Could you check a few things on this model? Use its own coordinates, in mm. Face numbers are marked on the shaded views. A direction names the side the tool comes from. Round coordinates to 2 decimals unless told otherwise and drop trailing zeros. Write each loop counter-clockwise with the first axis right and the second up, starting at its lowest first coordinate (ties: lowest second). Pieces come first, ordered by that corner, then holes. Notation, with made-up numbers: (54.5, -14) -> (64.5, -14) arc R17 ccw to (64.5, -7) -> close; hole circle Ø2 at (31.5, 70). An arc over 180 degrees is marked (long way). Answer in a Markdown table with one row per item. Add a question column.
```python
from build123d import *

# Parameters (mm, degrees)
BRACKET_BODY_DEPTH     = 50
POCKET_SKETCH_W        = 8
POCKET_SKETCH_H        = 60
POCKET_60X30_DEPTH     = 433.810582126
RAISED_PAD_SKETCH_R    = 25
RAISED_PAD_5MM_DEPTH   = 5
PAD_HOLE_SKETCH_R      = 10
PAD_HOLES_DEPTH        = 328.146756059
MOUNTING_HOLE_SKETCH_R = 7.25
MOUNTING_HOLES_DEPTH   = 25
THROUGH_HOLE_SKETCH_R  = 8
THROUGH_HOLES_16_DEPTH = 20
SADDLE_BLOCK_DEPTH     = 55
PIPE_SADDLE_CUT_DEPTH  = 55
SUPPORT_ARM_DEPTH      = 25
SUPPORT_WEB_15MM_DEPTH = 7.5


with BuildPart() as part:
    # Bracket Profile Sketch → Bracket Body (new, symmetric)
    with BuildSketch(Plane.XY):
        with BuildLine():
            Line((0, 110), (0, -250))
            Line((0, -250), (-25, -250))
            Line((-25, -250), (-25, -45))
            ThreePointArc((-25, -45), (-30.857864376, -30.857864376), (-45, -25))
            Line((-45, -25), (-235, -25))
            Line((-235, -25), (-235, 0))
            Line((-235, 0), (-45, 0))
            ThreePointArc((-45, 0), (-30.857864376, 5.857864376), (-25, 20))
            Line((-25, 20), (-25, 110))
            Line((-25, 110), (0, 110))
        make_face()
    extrude(amount=BRACKET_BODY_DEPTH, both=True)

    # Pocket Sketch → Pocket 60x30 (cut, through all)
    with BuildSketch(Plane(origin=(0, 110, 0), x_dir=(1, 0, 0), z_dir=(0, 1, 0))):
        with Locations((-4, 0)):
            Rectangle(POCKET_SKETCH_W, POCKET_SKETCH_H)
    extrude(amount=-POCKET_60X30_DEPTH, mode=Mode.SUBTRACT)

    # Raised Pad Sketch → Raised Pad 5mm (add)
    with BuildSketch(Plane.ZY.offset(25)):
        with Locations(Location((0, 75, 0), (0, 0, 90))):
            Circle(RAISED_PAD_SKETCH_R)
        with Locations(Location((0, -215, 0), (0, 0, 180))):
            Circle(RAISED_PAD_SKETCH_R)
    extrude(amount=RAISED_PAD_5MM_DEPTH)

    # Pad Hole Sketch → Pad Holes (cut, through all)
    with BuildSketch(Plane.ZY.offset(30)):
        with Locations(Location((0, 75, 0), (0, 0, 270))):
            Circle(PAD_HOLE_SKETCH_R)
        with Locations(Location((0, -215, 0), (0, 0, 270))):
            Circle(PAD_HOLE_SKETCH_R)
    extrude(amount=-PAD_HOLES_DEPTH, mode=Mode.SUBTRACT)

    # Mounting Hole Sketch → Mounting Holes (cut)
    with BuildSketch(Plane(origin=(0, 0, 0), x_dir=(1, 0, 0), z_dir=(0, 1, 0))):
        with Locations(Location((-75, 0, 0), (0, 0, 270))):
            Circle(MOUNTING_HOLE_SKETCH_R)
        with Locations(Location((-215, 0, 0), (0, 0, 270))):
            Circle(MOUNTING_HOLE_SKETCH_R)
    extrude(amount=-MOUNTING_HOLES_DEPTH, mode=Mode.SUBTRACT)

    # Through Hole Sketch → Through Holes Ø16 (cut)
    with BuildSketch(Plane(origin=(0, 0, 0), x_dir=(1, 0, 0), z_dir=(0, 1, 0))):
        with Locations(Location((-75, 0, 0), (0, 0, 270))):
            Circle(THROUGH_HOLE_SKETCH_R)
        with Locations(Location((-215, 0, 0), (0, 0, 270))):
            Circle(THROUGH_HOLE_SKETCH_R)
    extrude(amount=-THROUGH_HOLES_16_DEPTH, mode=Mode.SUBTRACT)

    # Saddle Block Sketch → Saddle Block (add, symmetric)
    with BuildSketch(Plane.XY):
        with BuildLine():
            Line((-194.749371855, 0), (-95.250628145, 0))
            ThreePointArc((-95.250628145, 0), (-145, -55), (-194.749371855, 0))
        make_face()
    extrude(amount=SADDLE_BLOCK_DEPTH, both=True)

    # Pipe Saddle Cut Sketch → Pipe Saddle Cut (cut, symmetric)
    with BuildSketch(Plane.XY):
        with BuildLine():
            Line((-190, 0), (-100, 0))
            Line((-100, 0), (-100, -5))
            Line((-100, -5), (-105, -5))
            ThreePointArc((-105, -5), (-145, -45), (-185, -5))
            Line((-185, -5), (-190, -5))
            Line((-190, -5), (-190, 0))
        make_face()
    extrude(amount=PIPE_SADDLE_CUT_DEPTH, both=True, mode=Mode.SUBTRACT)

    # Support Arm Sketch → Support Arm (add, symmetric)
    with BuildSketch(Plane.XY):
        with BuildLine():
            Line((-41.449496417, -158.46530057), (-175.781812899, -109.572335871))
            ThreePointArc((-175.781812899, -109.572335871), (-218.723683986, -76.621879272), (-235, -25))
            Line((-235, -25), (-219.833147735, -25))
            ThreePointArc((-219.833147735, -25), (-223.484631452, -26.584349745), (-224.822024251, -30.333333333))
            ThreePointArc((-224.822024251, -30.333333333), (-208.965317539, -73.046208509), (-172.361611466, -100.175409663))
            Line((-172.361611466, -100.175409663), (-42.446261863, -147.460729893))
            ThreePointArc((-42.446261863, -147.460729893), (-30.543506327, -145.893702398), (-25, -135.244725822))
            Line((-25, -135.244725822), (-25, -181.95761609))
            ThreePointArc((-25, -181.95761609), (-29.521198893, -167.618205181), (-41.449496417, -158.46530057))
        make_face()
    extrude(amount=SUPPORT_ARM_DEPTH, both=True)

    # Support Web Sketch → Support Web 15mm (add, symmetric)
    with BuildSketch(Plane.XY):
        with BuildLine():
            Line((-25, -45), (-25, -135.244725822))
            ThreePointArc((-25, -135.244725822), (-30.543506327, -145.893702398), (-42.446261863, -147.460729893))
            Line((-42.446261863, -147.460729893), (-172.361611466, -100.175409663))
            ThreePointArc((-172.361611466, -100.175409663), (-208.965317539, -73.046208509), (-224.822024251, -30.333333333))
            ThreePointArc((-224.822024251, -30.333333333), (-223.484631452, -26.584349745), (-219.833147735, -25))
            Line((-219.833147735, -25), (-190.82575695, -25))
            ThreePointArc((-190.82575695, -25), (-145, -55), (-99.17424305, -25))
            Line((-99.17424305, -25), (-45, -25))
            ThreePointArc((-45, -25), (-30.857864376, -30.857864376), (-25, -45))
        make_face()
    extrude(amount=SUPPORT_WEB_15MM_DEPTH, both=True)


solid = part.part
```
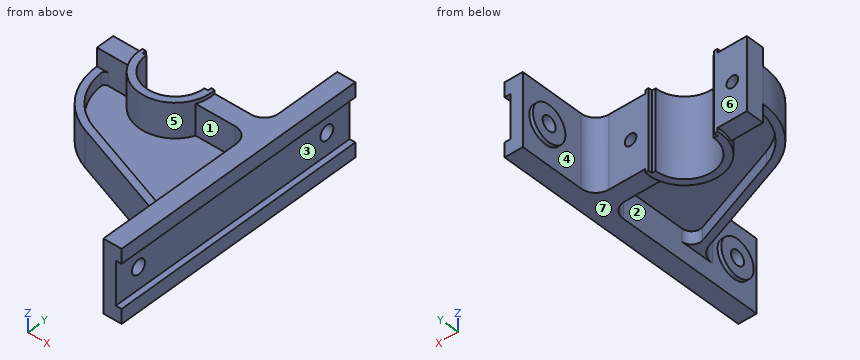
(1) I need wall thicknesses on L1, parallel to X at y = -4.75, z = 0; L2, parallel to Z at x = -215, y = -21.65; L3, parallel to X at y = -22.2, z = 0. Which ranges of each line are inside material? Lowest first, please.
(2) For P1, Ø8, axis at x = -190, z = 7, coming from the +Y side; P2, Ø1.5, axis at y = 30.5, z = 10.5, coming from the -X side; P3, Ø6, axis at x = -177.5, z = -32.5, coming from the +Y side, each with a flat end and sliding along its axis, tell me the tip position at first contact or that it passes through.
(3) On a 3-axis mill with a long thin cutter (end or side, diameter ignored), from which of +Z, -Z, +X, -X, +Y, -Y can I reach the whole of each face in a straight line? I mean the marked faces 1, 2 and 3. Say none if no direction works.
(4) Suppose I cut it at D-D, the plane x = -161. Please give me the cut outline in (y, z).
(5) Suppose I cut it at C-C, the plane y = 37. Please give me the cut outline in (x, z), then the cut area to 3 significant figures.
(6) If we mould it in two halves opening along Y, with no side actions, what happens to the marked faces 4, 5, 6 and 7? For each: pulls with the +Y half, pulls with the -Y half, needs draft (parallel to the pull), parting line crosses it, or undercut.
(7) Suppose I cut it at A-A, the plane y = -215. Please give me the cut outline in (x, z).
Response:
| question | item | result |
|---|---|---|
| 1 | L1 | -235 to -223, -207 to -190, -100 to -83, -67 to -8 |
| 1 | L2 | -50 to -7.25, 7.25 to 50 |
| 1 | L3 | -235 to -222.25, -207.75 to -181.11, -108.89 to -82.25, -67.75 to -8 |
| 2 | P1 | y = 0 |
| 2 | P2 | x = -25 |
| 2 | P3 | y = -23.43 |
| 3 | face 1 | +Z |
| 3 | face 2 | none |
| 3 | face 3 | +X, +Y, -Y |
| 4 | outline | (-114.95, -25) -> (-104.31, -25) -> (-104.31, -7.5) -> (-52.37, -7.5) -> (-52.37, -55) -> (-41.66, -55) -> (-41.66, 55) -> (-52.37, 55) -> (-52.37, 7.5) -> (-104.31, 7.5) -> (-104.31, 25) -> (-114.95, 25) -> close |
| 5 | outline | (-25, -50) -> (0, -50) -> (0, -30) -> (-8, -30) -> (-8, 30) -> (0, 30) -> (0, 50) -> (-25, 50) -> close |
| 5 | area | 2,020 mm² |
| 6 | face 4 | undercut |
| 6 | face 5 | undercut |
| 6 | face 6 | pulls with the +Y half |
| 6 | face 7 | needs draft |
| 7 | outline | (-30, -25) -> (-25, -25) -> (-25, -50) -> (0, -50) -> (0, -30) -> (-8, -30) -> (-8, -10) -> (-30, -10) -> close; (-30, 10) -> (-8, 10) -> (-8, 30) -> (0, 30) -> (0, 50) -> (-25, 50) -> (-25, 25) -> (-30, 25) -> close |
